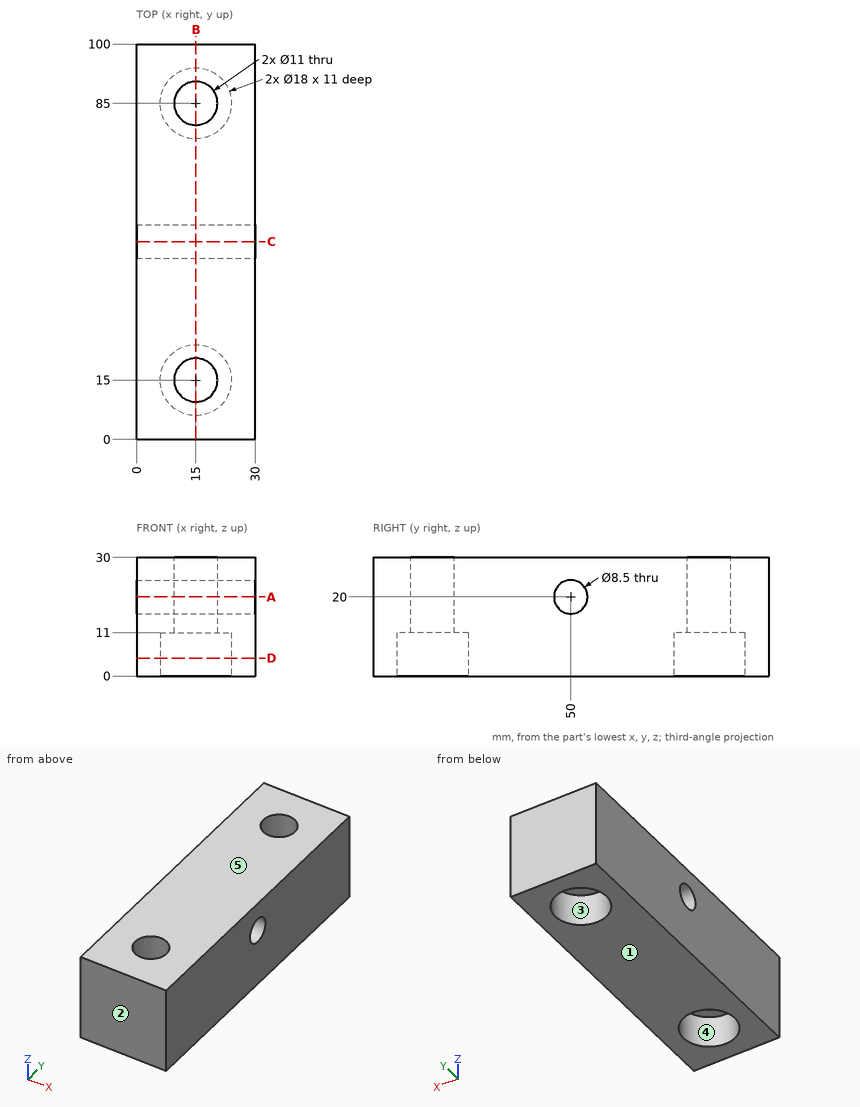
Source: three-view drawing plus pictorial views. Frame: mm from the lowest corner of the part. A direction names the side the tool comes from. Round coordinates to 2 decimals unless told otherwise and drop trailing zeros. Write each loop counter-clockwise with the first axis right and the second up, starting at its lowest first coordinate (ties: lowest second). Pieces come first, ordered by that corner, then holes. Notation, with made-up numbers: (-18.75, 15) -> (29.25, 15) arc R27 cw to (29.25, 43) -> close; hole circle Ø11 at (65.5, 15.5). An arc over 180 degrees is marked (long way). Return JSON: item names as keys, results as strings.
Q1. Section D-D on z = 4.5. Return the cut outline in (x, y), and give its area (3 significant figures).
From the geometry:
{"outline": "(0, 0) -> (30, 0) -> (30, 100) -> (0, 100) -> close; hole circle Ø18 at (15, 15); hole circle Ø18 at (15, 85)", "area": "2,490 mm2"}
Q2. First-contact query: pin 1 Ø14.5 at (x, y) = (15, 85) entering from +Z; pin 2 Ø14.5 at (x, y) = (15, 85) entering from -Z. Flat tips, straight axial feed; report the tip coordinate or a pass-through.
From the geometry:
{"pin 1": "z = 30", "pin 2": "z = 11"}
Q3. Section A-A on z = 20. Return the cut outline in (x, y).
From the geometry:
{"outline": "(0, 0) -> (30, 0) -> (30, 45.75) -> (0, 45.75) -> close; (0, 54.25) -> (30, 54.25) -> (30, 100) -> (0, 100) -> close; hole circle Ø11 at (15, 15); hole circle Ø11 at (15, 85)"}
Q4. Mould query, pull axis Y, two halves, no side actions, for the marked faces 1, 2 and 3. Classes: +Y half, -Y half, draft (parallel to the pull), parting line (faces both ways), or undercut.
From the geometry:
{"face 1": "draft", "face 2": "-Y half", "face 3": "undercut"}
Q5. Section B-B on x = 15. Return the cut outline in (y, z).
From the geometry:
{"outline": "(0, 0) -> (6, 0) -> (6, 11) -> (9.5, 11) -> (9.5, 30) -> (0, 30) -> close; (20.5, 11) -> (24, 11) -> (24, 0) -> (76, 0) -> (76, 11) -> (79.5, 11) -> (79.5, 30) -> (20.5, 30) -> close; (90.5, 11) -> (94, 11) -> (94, 0) -> (100, 0) -> (100, 30) -> (90.5, 30) -> close; hole circle Ø8.5 at (50, 20)"}
Q6. Section C-C on y = 50. Return the cut outline in (x, z).
From the geometry:
{"outline": "(0, 0) -> (30, 0) -> (30, 15.75) -> (0, 15.75) -> close; (0, 24.25) -> (30, 24.25) -> (30, 30) -> (0, 30) -> close"}
Q7. Set-up query: the marked faces 4 and 5. Return all of +Z, -Z, +X, -X, +Y, -Y with unobstructed straight access to the full face (end or side cutting, diameter ignored); none if empty.
From the geometry:
{"face 4": "-Z", "face 5": "+Z, +X, -X, +Y, -Y"}
Q8. Ray query, line 1 (Y direction, x = 15, z = 3.75); line 2 (Y direction, x = 12, z = 5.75); line 3 (Y direction, x = 15, z = 17.5). Return the intervals inside material, ascending.
From the geometry:
{"line 1": "0 to 6, 24 to 76, 94 to 100", "line 2": "0 to 6.51, 23.49 to 76.51, 93.49 to 100", "line 3": "0 to 9.5, 20.5 to 46.56, 53.44 to 79.5, 90.5 to 100"}
